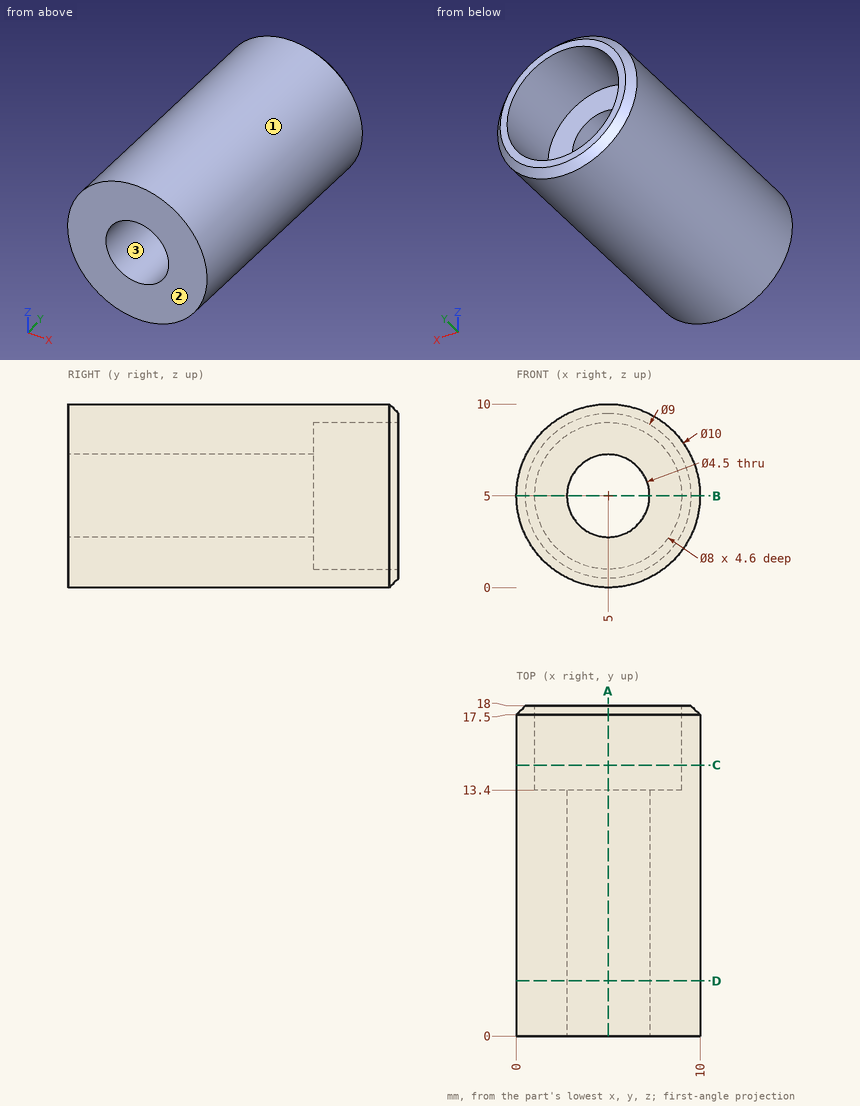
Study the drawing (mm; zero at the part's minimum x, y, z) and answer. Give positions to 0.01 mm unless a question says otherwise; leave off trailing zeros. Write each loop counter-clockwise with the first axis right and the second up, starting at its lowest first coordinate (ties: lowest second). Pieces come first, ordered by that corner, then holes. Notation, with made-up numbers: (13.5, -2) -> (35.5, -2) arc R13 cw to (35.5, 2) -> close; hole circle Ø5 at (40.5, -26). An arc over 180 degrees is marked (long way). Answer as a JSON object with one key per item and string values. Group by question number.
1) The mould has two halves that part along X. Classify the marked faces 1, 2 and 3: +X half, -X half, draft (parallel to the pull), parting line (faces both ways), or undercut.
2) This flat-tipped pin is pushed along its axis until it touches: P1, Ø2, axis at x = 2, y = 16, coming from the +Z side. Where does it stop, or does it pass through?
3) Find section A-A (x = 5). Write down the section's boundary in (y, z).
4) Find section C-C (y = 14.75). Write down the section's boundary in (x, z).
5) Consider L1, parallel to X at y = 10.5, z = 6; L2, parallel to Y at x = 7.75, z = 2.75; L3, parallel to Z at x = 8, y = 0.5. Determine where each line is inside the solid, lowest interval first. Write a range as from..to.
6) Find section D-D (y = 3). Write down the section's boundary in (x, z).
7) Find section B-B (z = 5). Write down the section's boundary in (x, y), and give its area (4 significant figures).
Values follow:
{
 "1": {"face 1": "parting line", "face 2": "draft", "face 3": "undercut"},
 "2": {"P1": "stops at z = 9.58"},
 "3": {"outline": "(0, 0) -> (17.5, 0) -> (18, 0.5) -> (18, 1) -> (13.4, 1) -> (13.4, 2.75) -> (0, 2.75) -> close; (0, 7.25) -> (13.4, 7.25) -> (13.4, 9) -> (18, 9) -> (18, 9.5) -> (17.5, 10) -> (0, 10) -> close"},
 "4": {"outline": "circle Ø10 at (5, 5); hole circle Ø8 at (5, 5)"},
 "5": {"L1": "x = 0.1..2.98, 7.02..9.9", "L2": "y = 0..13.4", "L3": "z = 1..9"},
 "6": {"outline": "circle Ø10 at (5, 5); hole circle Ø4.5 at (5, 5)"},
 "7": {"outline": "(0, 0) -> (2.75, 0) -> (2.75, 13.4) -> (1, 13.4) -> (1, 18) -> (0.5, 18) -> (0, 17.5) -> close; (7.25, 0) -> (10, 0) -> (10, 17.5) -> (9.5, 18) -> (9, 18) -> (9, 13.4) -> (7.25, 13.4) -> close", "area": "82.65 mm2"}
}
